Geometry check sheet. Reference: the model listing, model coordinates, mm. A direction names the side the tool comes from. Round coordinates to 2 decimals unless told otherwise and drop trailing zeros. Order: outer loops, then holes, each group sorted by start corner. A loop starts at its lowest first (then second) coordinate and runs counter-clockwise, first axis right, second up. Notation, with made-up numbers: (63.25, 38) -> (112.25, 38) arc R36 ccw to (112.25, 75) -> close; hole circle Ø1 at (81.5, -35.5). An arc over 180 degrees is marked (long way). Use a Markdown table: item, result. Add a question column.
Item 1: Sectioned sample at D-D, the plane y = 6.5. State how many separate pieces and enclosed holes the cut face has, and give its area (3 significant figures).
Item 2: Sectioned sample at A-A, the plane x = 7. Record the cut outline in (y, z).
Item 3: Gauge pin test, flat ends, axial feed: pin 1 Ø1.5 at (x, z) = (10, 4) entering from -Y; pin 2 Ø4.5 at (y, z) = (3.5, 1.5) entering from -X; pin 3 Ø5.5 at (x, z) = (21, -3.5) entering from +Y. Record the tip position at first contact, or that the pin passes through.
Item 4: Mould release check, pull along X, two halves, no side actions. Record for faces 5 (the flat face through (3, 4, -9.5)), 6 (the flat face through (14.929, -7.347, 0.133)), 7 (the cylindrical face through (-0.62, 4.724, 7.213)): pulls with the +X half, pulls with the -X half, needs draft (parallel to the pull), parting line crosses it, or undercut.
Item 5: Sectioned sample at B-B, the plane z = 0. Record the cut outline in (x, y).
Item 6: Set-up check for faces 1 (the flat face through (23.87, -3.2, 8.53)), 2 (the flat face through (19.05, -3, 0)), 3 (the flat face through (5, -2, -5.08)), 4 (the flat face through (-12.7, 5, 0)): record each of +Z, -Z, +X, -X, +Y, -Y from which the full face is reachable in a straight line by a thin tool's end or side.
Item 7: Sectioned sample at C-C, the plane x = 26.04. Record the cut outline in (y, z) (3 decimals).
Item 8: Material ranges on probe 1 along Z at (x, y) = (6.5, 4.25); probe 2 along X at (y, z) = (-1.75, -6.5); probe 3 along X at (y, z) = (6.25, -6.5), recorded low to high. Write a range as [from, to].
from build123d import *
from OCP.BRepFilletAPI import BRepFilletAPI_MakeChamfer

# Parameters (mm, degrees)
ROCKER_BODY_PROFILE_SKETCH_R      = 4.765
ROCKER_BODY_DEPTH                 = 9.5
ARM_END_CHAMFER_A_SIZE            = 7.62
ARM_END_CHAMFER_A_SIZE2           = 2.54
ARM_END_CHAMFER_B_SIZE            = 2.54
ARM_END_CHAMFER_B_SIZE2           = 7.62
FORK_SLOTS_SKETCH_W               = 9.53
FORK_SLOTS_SKETCH_H               = 9.53
FORK_SLOT_CUT_A_DEPTH             = 32.662585176
FORK_SLOT_CUT_B_DEPTH             = 32.662585176
FORK_SLOT_CUT_B_DEPTH_BACK        = 32.662585176
SKETCH2_2_W                       = 9.53
SKETCH2_2_H                       = 9.53
CENTRE_POCKET_DEPTH               = 32.662585176
CENTRE_POCKET_DEPTH_BACK          = 32.662585176
FORK_PIN_HOLES_2X_3_18_DEPTH      = 32.662585236
FORK_PIN_HOLES_2X_3_18_DEPTH_BACK = 32.662585236
FORK_PIN_HOLES_SKETCH_R           = 1.59


with BuildPart() as part:
    # Rocker Body Profile Sketch → Rocker Body (new, symmetric)
    with BuildSketch(Plane.XY):
        with BuildLine():
            Line((0, 9.77), (-22.23, 9.77))
            Line((-22.23, 9.77), (-22.23, 4.77))
            Line((-22.23, 4.77), (-9.711509246, -1.067468107))
            ThreePointArc((-9.711509246, -1.067468107), (-5.877874817, -7.804068659), (1.655323868, -9.628748771))
            Line((1.655323868, -9.628748771), (28.58, -5))
            Line((28.58, -5), (28.58, 0))
            Line((28.58, 0), (9.77, 0))
            ThreePointArc((9.77, 0), (6.908433252, 6.908433252), (0, 9.77))
        make_face()
        Circle(ROCKER_BODY_PROFILE_SKETCH_R, mode=Mode.SUBTRACT)
    extrude(amount=ROCKER_BODY_DEPTH, both=True)

    # Arm End Chamfer A
    arm_end_chamfer_a_edges = [part.edges().sort_by_distance(p)[0] for p in [
        (-22.23, 7.27, -9.5),
        (28.58, -2.5, -9.5),
    ]]
    arm_end_chamfer_a_side = [part.faces().sort_by_distance(p)[0] for p in [
        (-11.115, 9.225622585, -9.5),
    ]]
    chamfer(arm_end_chamfer_a_edges, length=ARM_END_CHAMFER_A_SIZE, length2=ARM_END_CHAMFER_A_SIZE2, reference=arm_end_chamfer_a_side[0])

    # Arm End Chamfer B: one chamfer whose edges measure the first distance from different faces: ONE call of the kernel's chamfer builder (chamfer() names one face for all edges)
    arm_end_chamfer_b_edges_1 = [part.edges().sort_by_distance(p)[0] for p in [
        (-22.23, 7.27, 9.5),
    ]]
    arm_end_chamfer_b_side_1 = [part.faces().sort_by_distance(p)[0] for p in [
        (-22.23, 7.27, 1.27),
    ]]
    arm_end_chamfer_b_edges_2 = [part.edges().sort_by_distance(p)[0] for p in [
        (28.58, -2.5, 9.5),
    ]]
    arm_end_chamfer_b_side_2 = [part.faces().sort_by_distance(p)[0] for p in [
        (28.58, -2.5, 1.27),
    ]]
    arm_end_chamfer_b = BRepFilletAPI_MakeChamfer(part.part.solid().wrapped)
    for e in arm_end_chamfer_b_edges_1:
        arm_end_chamfer_b.Add(ARM_END_CHAMFER_B_SIZE, ARM_END_CHAMFER_B_SIZE2, e.wrapped, arm_end_chamfer_b_side_1[0].wrapped)  # the first distance lies on this face
    for e in arm_end_chamfer_b_edges_2:
        arm_end_chamfer_b.Add(ARM_END_CHAMFER_B_SIZE, ARM_END_CHAMFER_B_SIZE2, e.wrapped, arm_end_chamfer_b_side_2[0].wrapped)  # the first distance lies on this face
    add(Compound.cast(arm_end_chamfer_b.Shape()), mode=Mode.REPLACE)

    # Fork Slots Sketch → Fork Slot Cut A (cut, through all)
    with BuildSketch(Plane(origin=(0, 0, 0), x_dir=(1, 0, 0), z_dir=(0, 1, 0))):
        with Locations((-17.465, 0)):
            Rectangle(FORK_SLOTS_SKETCH_W, FORK_SLOTS_SKETCH_H)
        with Locations((23.815, 0)):
            Rectangle(FORK_SLOTS_SKETCH_W, FORK_SLOTS_SKETCH_H)
    extrude(amount=-FORK_SLOT_CUT_A_DEPTH, mode=Mode.SUBTRACT)

    # Sketch2_2 → Fork Slot Cut B (cut, two sides: drawn at the far end of the back side and taken through both)
    with BuildSketch(Plane(origin=(0, 0, 0), x_dir=(1, 0, 0), z_dir=(0, 1, 0)).offset(-FORK_SLOT_CUT_B_DEPTH_BACK)):
        with Locations((-17.465, 0)):
            Rectangle(SKETCH2_2_W, SKETCH2_2_H)
        with Locations((23.815, 0)):
            Rectangle(SKETCH2_2_W, SKETCH2_2_H)
    extrude(amount=FORK_SLOT_CUT_B_DEPTH + FORK_SLOT_CUT_B_DEPTH_BACK, mode=Mode.SUBTRACT)

    # Centre Pocket Sketch → Centre Pocket (cut, two sides: drawn at the far end of the back side and taken through both)
    with BuildSketch(Plane(origin=(0, 0, 0), x_dir=(1, 0, 0), z_dir=(0, 1, 0)).offset(-CENTRE_POCKET_DEPTH_BACK)):
        with BuildLine():
            Line((-3.81, 5.08), (6.35, 5.08))
            ThreePointArc((6.35, 5.08), (11.43, 0), (6.35, -5.08))
            Line((6.35, -5.08), (-3.81, -5.08))
            ThreePointArc((-3.81, -5.08), (-8.89, 0), (-3.81, 5.08))
        make_face()
    extrude(amount=CENTRE_POCKET_DEPTH + CENTRE_POCKET_DEPTH_BACK, mode=Mode.SUBTRACT)

    # Fork Pin Holes Sketch → Fork Pin Holes 2x_3.18 (cut, two sides: drawn at the far end of the back side and taken through both)
    with BuildSketch(Plane.XY.offset(-FORK_PIN_HOLES_2X_3_18_DEPTH_BACK)):
        with Locations((-19.69, 7.23)):
            Circle(FORK_PIN_HOLES_SKETCH_R)
        with Locations((26.04, -2.54)):
            Circle(FORK_PIN_HOLES_SKETCH_R)
    extrude(amount=FORK_PIN_HOLES_2X_3_18_DEPTH + FORK_PIN_HOLES_2X_3_18_DEPTH_BACK, mode=Mode.SUBTRACT)


solid = part.part
Found:
| question | item | result |
|---|---|---|
| 1 | separate pieces | 3 |
| 1 | enclosed holes | 0 |
| 1 | area | 280 mm2 |
| 2 | outline | (-8.71, -9.5) -> (6.82, -9.5) -> (6.82, -5.04) -> (-8.71, -5.04) -> close; (-8.71, 5.04) -> (6.82, 5.04) -> (6.82, 9.5) -> (-8.71, 9.5) -> close |
| 3 | pin 1 | stops at y = -8.32 |
| 3 | pin 2 | stops at x = -12.7 |
| 3 | pin 3 | stops at y = 0 |
| 4 | face 5 | needs draft |
| 4 | face 6 | pulls with the +X half |
| 4 | face 7 | undercut |
| 5 | outline | (-12.7, 0.33) -> (-9.71, -1.07) arc R9.77 ccw to (-8.89, -4.05) -> (-8.89, 9.77) -> (-12.7, 9.77) -> close; (11.43, -7.95) -> (19.05, -6.64) -> (19.05, 0) -> (11.43, 0) -> close |
| 6 | face 1 | +Z, +X, +Y, -Y |
| 6 | face 2 | +X, +Y, -Y |
| 6 | face 3 | +Y, -Y |
| 6 | face 4 | -X, +Y, -Y |
| 7 | outline | (-5.437, -7.807) -> (-4.13, -7.807) -> (-4.13, -4.765) -> (-5.437, -4.765) -> close; (-5.437, 4.765) -> (-4.13, 4.765) -> (-4.13, 7.807) -> (-5.437, 7.807) -> close; (-0.95, -7.807) -> (0, -7.807) -> (0, -4.765) -> (-0.95, -4.765) -> close; (-0.95, 4.765) -> (0, 4.765) -> (0, 7.807) -> (-0.95, 7.807) -> close |
| 8 | probe 1 | z = [-9.5, -5.08], [5.08, 9.5] |
| 8 | probe 2 | x = [-9.61, -4.43], [4.43, 24.66], [27.42, 28.58] |
| 8 | probe 3 | x = [-22.23, -20.94], [-18.44, 7.51] |
